For this review, take the finished solid that the model builds, in its own axes (mm). A direction names the side the tool comes from. Give positions to 0.01 mm unless a question says otherwise; leave off trailing zeros. Loops run counter-clockwise (first coordinate to the right, second up) from the corner with the lowest first, then second, coordinate; pieces in that order, holes last. Notation, with made-up numbers: (35.5, -30) - (58.5, -30) arc R24 cw to (58.5, -13) - close; hole circle Ø10 at (12.5, 53.25). An arc over 180 degrees is marked (long way). Use CSV: the item, a comma, the result in double quotes. Start each with the question number.
1. Take a section at B-B on x = -1216. Give the boundary of the cut face in (y, z), plus the area to 3 significant figures.
2. Take a section at A-A on z = 30.5. Give the boundary of the cut face in (x, y).
3. For faces 4 (the flat face through (-215, 19.409, 39)), 5 (the flat face through (-814, -98, 0)), list the 3-axis set-ups (+Z, -Z, +X, -X, +Y, -Y) from which the entire face can be reached by the end or side of a thin tool; tool diameter is ignored.
4. Take a section at C-C on y = -112. Give the boundary of the cut face in (x, z).
5. For pin 1 (20 mm diameter, centred on y = 34.5, z = 44, fed in from -X); pin 2 (23.5 mm diameter, centred on x = -1010, z = 28.5, fed in from +Y); pin 3 (10 mm diameter, centred on y = -73.5, z = 62.5, fed in from -X); pin 4 (5.5 mm diameter, centred on x = -1887.9, z = 74, fed in from +Y), all flat-tipped, find the tip position at first contact; note any pin that passes through.
6. Take a section at D-D on y = 42. Give the boundary of the cut face in (x, z).
7. Mouldability with a two-part tool opening along Y and no side actions: class faces 1 (the flat face through (-211, 59.409, 39)), 2 (the flat face through (-327.901, 40, 39)), 3 (the cylindrical face through (-42.914, -34.381, 38.947)) as pulls with the +Y half, pulls with the -Y half, needs draft (parallel to the pull), parting line crosses it, or undercut.
8. Wall thickness on line 1 (X direction, y = 32, z = 74); line 2 (Y direction, x = -284.5, z = 13); line 3 (X direction, y = -38, z = 45): over which ranges is each line inside the solid? List them lowest first.
```python
from build123d import *

# Parameters (mm, degrees)
EXTRUDE_1_DEPTH           = 79
HOLE_WIZARD_7_0_7_1_D     = 7
HOLE_WIZARD_7_0_7_2_D     = 7
HOLE_WIZARD_7_0_7_2_DEPTH = 40


with BuildPart() as part:
    # 草图1 → 凸台-拉伸1 (new body)
    with BuildSketch(Plane.XY):
        with BuildLine():
            Line((-327.90073838, 19.409448819), (-97.90073838, 19.409448819))
            ThreePointArc((-97.90073838, 19.409448819), (-42.90073838, -35.590551181), (-97.90073838, -90.590551181))
            Line((-97.90073838, -90.590551181), (-1897.90073838, -90.590551181))
            Line((-1897.90073838, -90.590551181), (-1897.90073838, -130.590551181))
            Line((-1897.90073838, -130.590551181), (-97.90073838, -130.590551181))
            ThreePointArc((-97.90073838, -130.590551181), (-2.90073838, -35.590551181), (-97.90073838, 59.409448819))
            Line((-97.90073838, 59.409448819), (-327.90073838, 59.409448819))
            Line((-327.90073838, 59.409448819), (-327.90073838, 19.409448819))
        make_face()
    extrude(amount=EXTRUDE_1_DEPTH)

    # Ø7.0 (7) 直径孔1 (through all)
    with Locations(Plane(origin=(0, -130.590551181, 0), x_dir=(-1, 0, 0), z_dir=(0, -1, 0))):
        with Locations((1872.90073838, -5), (1887.90073838, -5), (1872.90073838, -74), (1887.90073838, -74)):
            Hole(HOLE_WIZARD_7_0_7_1_D / 2)

    # Ø7.0 (7) 直径孔2
    with Locations(Plane(origin=(0, 59.409448819, 0), x_dir=(1, 0, 0), z_dir=(0, 1, 0))):
        with Locations((-317.90073838, -5), (-302.90073838, -5), (-317.90073838, -74), (-302.90073838, -74)):
            Hole(HOLE_WIZARD_7_0_7_2_D / 2, depth=HOLE_WIZARD_7_0_7_2_DEPTH)


solid = part.part
```
Check result:
1,outline,"(-130.59, 0) - (-90.59, 0) - (-90.59, 79) - (-130.59, 79) - close"
1,area,"3,160 mm²"
2,outline,"(-1897.9, -130.59) - (-97.9, -130.59) arc R95 ccw to (-97.9, 59.41) - (-327.9, 59.41) - (-327.9, 19.41) - (-97.9, 19.41) arc R55 cw to (-97.9, -90.59) - (-1897.9, -90.59) - close"
3,face 4,"+Z, -Z, -X"
3,face 5,"-Z, +X, -X, +Y, -Y"
4,outline,"(-1897.9, 0) - (-41.45, 0) - (-41.45, 79) - (-1897.9, 79) - close; hole circle Ø7 at (-1887.9, 5); hole circle Ø7 at (-1887.9, 74); hole circle Ø7 at (-1872.9, 5); hole circle Ø7 at (-1872.9, 74)"
5,pin 1,"stops at x = -327.9"
5,pin 2,"stops at y = -90.59"
5,pin 3,"stops at x = -63.49"
5,pin 4,"passes through"
6,outline,"(-327.9, 0) - (-43.09, 0) - (-43.09, 79) - (-327.9, 79) - close; hole circle Ø7 at (-317.9, 5); hole circle Ø7 at (-317.9, 74); hole circle Ø7 at (-302.9, 5); hole circle Ø7 at (-302.9, 74)"
7,face 1,"pulls with the +Y half"
7,face 2,"needs draft"
7,face 3,"undercut"
8,line 1,"x = -327.9 to -321.4, -314.4 to -306.4, -299.4 to -31.14"
8,line 2,"y = -130.59 to -90.59, 19.41 to 59.41"
8,line 3,"x = -42.95 to -2.93"
